Design review of the part built by this model. Coordinates are the model's own, in mm. A direction names the side the tool comes from. Give positions to 0.01 mm unless a question says otherwise; leave off trailing zeros. Loops run counter-clockwise (first coordinate to the right, second up) from the corner with the lowest first, then second, coordinate; pieces in that order, holes last. Notation, with made-up numbers: M -36,66.25 L -28,66.25 A17 cw -28,95.25 Z; hole C -19,-21 d1. An arc over 180 degrees is marked long. Use a Markdown table: item, result. Add a question column.
(1) For probe 1 along Y at (x, z) = (39, 61); probe 2 along X at (y, z) = (1.2, 45), list the stretches that pass through material, from the lowest coordinate up.
(2) Add section A-A, the plane z = 45. Give the boundary of the cut face in (x, y).
(3) Draft analysis for pull direction Y (two halves, no side actions). For faces 1 (the face through (25, 0, 64)), 2 (the face through (47, 25, 64)), 3 (the face through (2.7, 25.1, 0)), 4 (the face through (25, 50, 64)), state which applies: pulls with the +Y half, pulls with the -Y half, needs draft (parallel to the pull), parting line crosses it, or undercut.
(4) Add section B-B, the plane x = 25. Give the boundary of the cut face in (y, z).
(5) Add section C-C, the plane y = 8. Give the boundary of the cut face in (x, z).
(6) For faces 5 (the face through (25, 3, 64)), 6 (the face through (50, 25, 64)), list the 3-axis set-ups (+Z, -Z, +X, -X, +Y, -Y) from which the entire face can be reached by the end or side of a thin tool; tool diameter is ignored.
(7) Insertion check: pin 1 Ø8 at (x, y) = (40, 39) entering from -Z. The pin has a flat end and moves straight along its axis. Give the tip position at first contact, or say it passes through.
(8) Add section D-D, the plane z = 85. Give the boundary of the cut face in (x, y), then the cut area to 3 significant figures.
```python
from build123d import *

# Parameters (mm, degrees)
SKETCH_1_W          = 50
SKETCH_1_H          = 50
SKETCH_1_W_2        = 44
SKETCH_1_H_2        = 44
EXTRUDE_1_DEPTH     = 130
SKETCH_5_R          = 6.5
CUT_EXTRUDE_1_DEPTH = 130


with BuildPart() as part:
    # 草图1 → 凸台-拉伸1 (new body)
    with BuildSketch(Plane.XY):
        with Locations((25, 25)):
            Rectangle(SKETCH_1_W, SKETCH_1_H)
        with Locations((25, 25)):
            Rectangle(SKETCH_1_W_2, SKETCH_1_H_2, mode=Mode.SUBTRACT)
    extrude(amount=EXTRUDE_1_DEPTH)

    # 草图5 → 切除-拉伸1 (cut)
    with BuildSketch(Plane(origin=(0, 50, 0), x_dir=(1, 0, 0), z_dir=(0, 1, 0))):
        with Locations(Location((25, -45, 0), (0, 0, 270))):
            Circle(SKETCH_5_R)
    extrude(amount=-CUT_EXTRUDE_1_DEPTH, mode=Mode.SUBTRACT)


solid = part.part
```
Established:
| question | item | result |
|---|---|---|
| 1 | probe 1 | 0 to 3, 47 to 50 |
| 1 | probe 2 | 0 to 18.5, 31.5 to 50 |
| 2 | outline | M 0,0 L 18.5,0 L 18.5,3 L 3,3 L 3,47 L 18.5,47 L 18.5,50 L 0,50 Z; M 31.5,0 L 50,0 L 50,50 L 31.5,50 L 31.5,47 L 47,47 L 47,3 L 31.5,3 Z |
| 3 | face 1 | pulls with the -Y half |
| 3 | face 2 | undercut |
| 3 | face 3 | needs draft |
| 3 | face 4 | pulls with the +Y half |
| 4 | outline | M 0,0 L 3,0 L 3,38.5 L 0,38.5 Z; M 0,51.5 L 3,51.5 L 3,130 L 0,130 Z; M 47,0 L 50,0 L 50,38.5 L 47,38.5 Z; M 47,51.5 L 50,51.5 L 50,130 L 47,130 Z |
| 5 | outline | M 0,0 L 3,0 L 3,130 L 0,130 Z; M 47,0 L 50,0 L 50,130 L 47,130 Z |
| 6 | face 5 | +Z, -Z |
| 6 | face 6 | +Z, -Z, +X, +Y, -Y |
| 7 | pin 1 | through |
| 8 | outline | M 0,0 L 50,0 L 50,50 L 0,50 Z; hole M 3,3 L 47,3 L 47,47 L 3,47 Z |
| 8 | area | 564 mm^2 |
